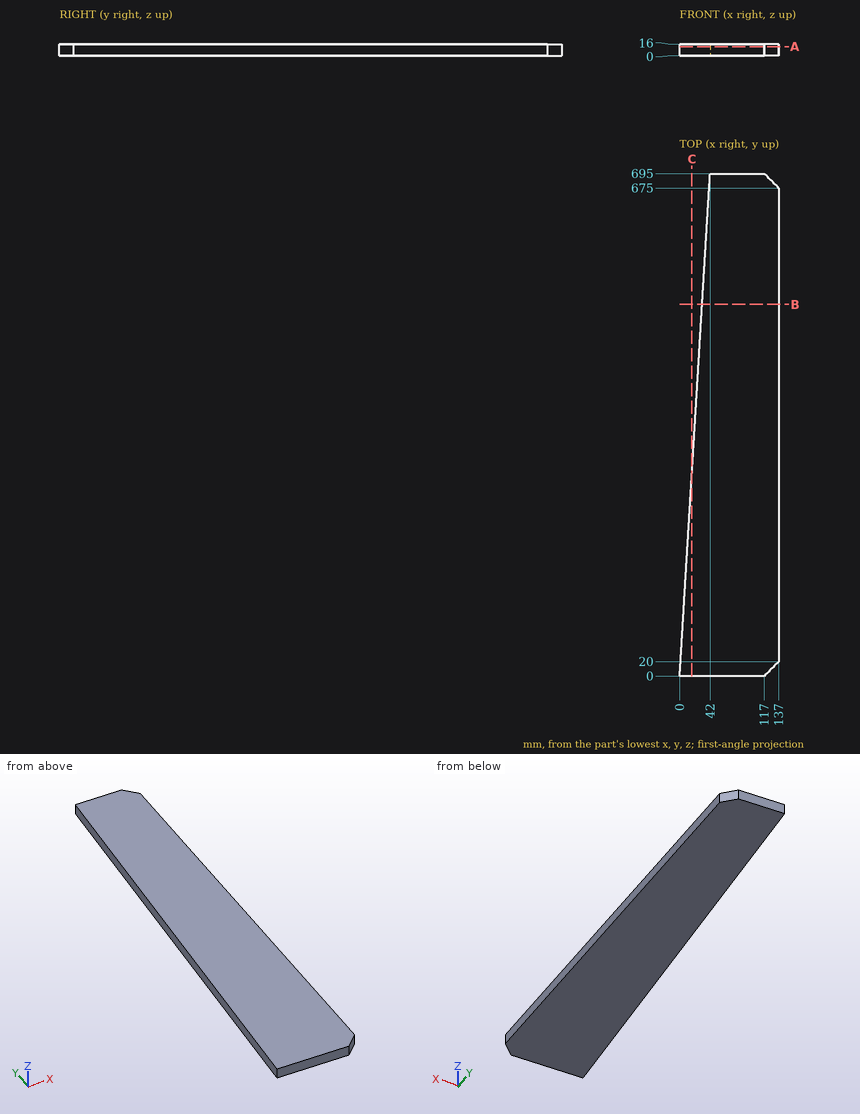
Geometry check sheet. Reference: drawing and pictorial views, mm from the part's lowest x, y, z. Round coordinates to 2 decimals unless told otherwise and drop trailing zeros. Loops run counter-clockwise (first coordinate to the right, second up) from the corner with the lowest first, then second, coordinate; pieces in that order, holes last. Notation, with made-up numbers: (-13, -2) -> (26, -2) arc R10 cw to (26, 9) -> close; hole circle Ø9 at (86.5, -15.5). An arc over 180 degrees is marked (long way). Answer as a JSON object with one key per item and string values. Group by question number.
Item 1: Cross-section at C-C, the plane x = 17. Record the cut outline in (y, z).
Item 2: Depth check by flat-ended pin: pin 1 Ø5 at (y, z) = (489.5, 5) entering from -X. Enter the tip coordinate at first touch or a pass-through.
Item 3: Cross-section at B-B, the plane y = 514. Record the cut outline in (x, z).
Item 4: Thickness scan on line 1 along X through (y, z) = (225, 4.75); line 2 along X through (y, z) = (381.5, 11.25); line 3 along Y through (x, z) = (120, 12.25). Record the ranges inside material, lowest first.
Item 5: Cross-section at A-A, the plane z = 12.25. Record the cut outline in (x, y).
Determined:
{
 "1": {"outline": "(0, 0) -> (281.31, 0) -> (281.31, 16) -> (0, 16) -> close"},
 "2": {"pin 1": "stops at x = 29.43"},
 "3": {"outline": "(31.06, 0) -> (137, 0) -> (137, 16) -> (31.06, 16) -> close"},
 "4": {"line 1": "x = 13.6 to 137", "line 2": "x = 23.05 to 137", "line 3": "y = 3 to 692"},
 "5": {"outline": "(0, 0) -> (117, 0) -> (137, 20) -> (137, 675) -> (117, 695) -> (42, 695) -> close"}
}
